```python
from build123d import *

# Parameters (mm, degrees)
SKETCH7_OUTSIDE_W   = 84.804
SKETCH7_OUTSIDE_H   = 84.804
SKETCH7_OUTSIDE_W_2 = 34
SKETCH7_OUTSIDE_H_2 = 45
CUT_EXTRUDE3_DEPTH  = 25
M4_TAPPED_HOLE2_D   = 3.3
SKETCH13_R          = 2
CUT_EXTRUDE6_DEPTH  = 25
SKETCH14_R          = 5.5
CUT_EXTRUDE7_DEPTH  = 151.66270275
CHAMFER1_SIZE       = 0.2
CHAMFER2_SIZE       = 0.5
SKETCH15_W          = 4.842021814
SKETCH15_H          = 7.203372967
CUT_EXTRUDE8_DEPTH  = 5
CUT_EXTRUDE9_DEPTH  = 154.513028763
SKETCH17_W          = 3.088959923
SKETCH17_H          = 8.04850145
SKETCH17_W_2        = 2.99848013
SKETCH17_H_2        = 8.967280155
CUT_EXTRUDE10_DEPTH = 5


with BuildPart() as part:
    # Sketch1 → Revolve1 (revolve)
    with BuildSketch(Plane.XY, mode=Mode.PRIVATE) as revolve1_sk:
        Polygon((0, 0), (11, 0), (11, 12), (25, 12), (25, 24), (17, 24), (17, 29), (12.5, 29), (12.5, 84), (10, 84), (10, 94), (9.5, 94), (9.5, 129), (8.5, 129), (8.5, 137), (8, 137), (8, 138.1), (8.5, 138.1), (8.5, 148), (0, 148), align=None)
    revolve(revolve1_sk.sketch.rotate(Axis((0, 148, 0), (0, -1, 0)), 90), axis=Axis((0, 148, 0), (0, -1, 0)))

    # Sketch7 outside → Cut-Extrude3 (cut)
    with BuildSketch(Plane(origin=(0, 24, 0), x_dir=(1, 0, 0), z_dir=(0, 1, 0))):
        Rectangle(SKETCH7_OUTSIDE_W, SKETCH7_OUTSIDE_H)
        Rectangle(SKETCH7_OUTSIDE_W_2, SKETCH7_OUTSIDE_H_2, mode=Mode.SUBTRACT)
    extrude(amount=-CUT_EXTRUDE3_DEPTH, mode=Mode.SUBTRACT)

    # M4 Tapped Hole2 (through all)
    with Locations(Plane(origin=(0, 12, 0), x_dir=(-1, 0, 0), z_dir=(0, -1, 0))):
        with Locations((-12.5, 17.5), (12.5, -17.5)):
            Hole(M4_TAPPED_HOLE2_D / 2)

    # Sketch13 → Cut-Extrude6 (cut)
    with BuildSketch(Plane.XZ.offset(-12)):
        with Locations(Location((12.5, 17.5, 0), (0, 0, 270))):
            Circle(SKETCH13_R)
        with Locations(Location((-12.5, -17.5, 0), (0, 0, 270))):
            Circle(SKETCH13_R)
    extrude(amount=-CUT_EXTRUDE6_DEPTH, mode=Mode.SUBTRACT)

    # Sketch14 → Cut-Extrude7 (cut, through all)
    with BuildSketch(Plane.XZ):
        Circle(SKETCH14_R)
    extrude(amount=-CUT_EXTRUDE7_DEPTH, mode=Mode.SUBTRACT)

    # Chamfer1
    chamfer1_edges = [part.edges().sort_by_distance(p)[0] for p in [
        (0, 148, -8.5),
        (0, 84, -12.5),
    ]]
    chamfer(chamfer1_edges, length=CHAMFER1_SIZE)

    # Chamfer2
    chamfer2_edges = [part.edges().sort_by_distance(p)[0] for p in [
        (-5.5, 148, 0),
        (-5.5, 0, 0),
        (0, 0, -11),
    ]]
    chamfer(chamfer2_edges, length=CHAMFER2_SIZE)

    # Sketch15 → Cut-Extrude8 (cut, symmetric)
    with BuildSketch(Plane.XY):
        with Locations((10.421010907, 146.101686484)):
            Rectangle(SKETCH15_W, SKETCH15_H)
    extrude(amount=CUT_EXTRUDE8_DEPTH, both=True, mode=Mode.SUBTRACT)

    # Sketch16 → Cut-Extrude9 (cut, through all)
    with BuildSketch(Plane.ZY.offset(17)):
        with BuildLine():
            Line((-3, 21), (3, 21))
            ThreePointArc((3, 21), (6, 18), (3, 15))
            Line((3, 15), (-3, 15))
            ThreePointArc((-3, 15), (-6, 18), (-3, 21))
        make_face()
    extrude(amount=-CUT_EXTRUDE9_DEPTH, mode=Mode.SUBTRACT)

    # Sketch17 → Cut-Extrude10 (cut, symmetric)
    with BuildSketch(Plane(origin=(0, 0, 0), x_dir=(0, 0, -1), z_dir=(1, 0, 0))):
        with Locations((9.544479962, 146.524250725)):
            Rectangle(SKETCH17_W, SKETCH17_H)
        with Locations((-9.499240065, 146.983640078)):
            Rectangle(SKETCH17_W_2, SKETCH17_H_2)
    extrude(amount=CUT_EXTRUDE10_DEPTH, both=True, mode=Mode.SUBTRACT)


solid = part.part
```
The model under review builds one solid part; all positions refer to its coordinate system, in mm. A direction names the side the tool comes from. Round coordinates to 2 decimals unless told otherwise and drop trailing zeros. Write each loop counter-clockwise with the first axis right and the second up, starting at its lowest first coordinate (ties: lowest second). Pieces come first, ordered by that corner, then holes. Notation, with made-up numbers: (-4.75, 67.5) - (38.25, 67.5) arc R18 ccw to (38.25, 96.5) - close; hole circle Ø2 at (52, 35). An arc over 180 degrees is marked (long way). Use one line per item in the form item = value.
Q1. Insertion check: pin 1 Ø3 at (x, y) = (-7.5, 95) entering from +Z; pin 2 Ø2 at (x, z) = (12.5, -17.5) entering from +Y; pin 3 Ø4.5 at (y, z) = (146.5, -0.5) entering from +X; pin 4 Ø1 at (y, z) = (101, -1) entering from -X. Each pin has a flat end and moves straight along its axis. Give the tip position at first contact, or say it passes through.
Answer key:
pin_1 = 7.7
pin_2 = through
pin_3 = 8
pin_4 = -9.49
Q2. Draft analysis for pull direction Z (two halves, no side actions). For faces 4 (the flat face through (0, 145, -8)), 5 (the cylindrical face through (13.39, 18.08, -18.89)), 6 (the flat face through (-10, 84, -2)), state which applies: +Z half, -Z half, draft (parallel to the pull), parting line (faces both ways), or undercut.
Answer key:
face_4 = -Z half
face_5 = undercut
face_6 = draft
Q3. Consider section B-B (y = 63). State the section outline as (x, z) points.
Answer key:
outline = circle Ø25 at (0, 0); hole circle Ø11 at (0, 0)
Q4. Tool access review of faces 1 (the flat face through (8, 145, 0)), 2 (the flat face through (-12, 12, 0)), 3 (the cylindrical face through (-3.755, 56.784, 11.923)): name each direction out of +Z, -Z, +X, -X, +Y, -Y from which nothing blocks a thin tool from reaching the whole face with its end or side.
Answer key:
face_1 = +Z, -Z, +X, +Y
face_2 = -Y
face_3 = +Y
Q5. Consider section C-C (y = 117). State the section outline as (x, z) points, and give its area (3 significant figures).
Answer key:
outline = circle Ø19 at (0, 0); hole circle Ø11 at (0, 0)
area = 188 mm2
Q6. For line 1 (X direction, y = 9, z = 0); line 2 (X direction, y = 15, z = -17); line 3 (X direction, y = 73, z = 0), list the stretches that pass through material, from the lowest coordinate up. Write a range as [from, to].
Answer key:
line_1 = [-11, -5.5], [5.5, 11]
line_2 = [-17, -14.44], [-10.56, 10.93], [14.07, 17]
line_3 = [-12.5, -5.5], [5.5, 12.5]
Q7. Consider section A-A (y = 18). State the section outline as (x, z) points, and give its area (3 significant figures).
Answer key:
outline = (-17, -18.33) arc R25 ccw to (-10.9, -22.5) - (10.9, -22.5) arc R25 ccw to (17, -18.33) - (17, -6) - (-17, -6) - close; (-17, 6) - (17, 6) - (17, 18.33) arc R25 ccw to (10.9, 22.5) - (-10.9, 22.5) arc R25 ccw to (-17, 18.33) - close; hole circle Ø4 at (-12.5, -17.5); hole circle Ø3.3 at (-12.5, 17.5); hole circle Ø4 at (12.5, 17.5); hole circle Ø3.3 at (12.5, -17.5)
area = 1,030 mm2
